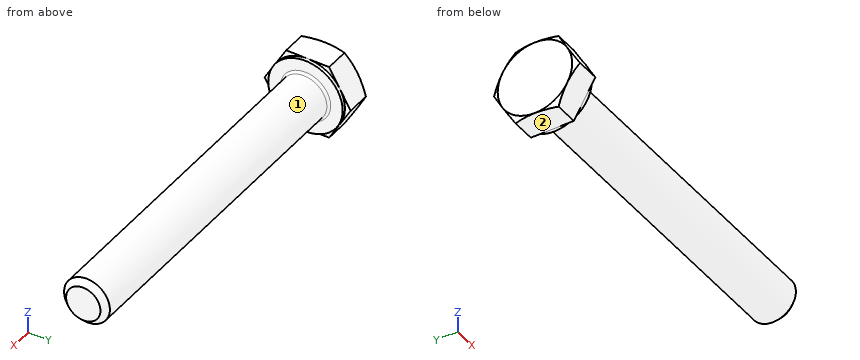
from build123d import *

# Parameters (mm, degrees)
BASE_EXTRUDE_DEPTH = 5.3
SKETCH4_W          = 0.6
SKETCH4_H          = 11.005553499
CHAMFER_2_SIZE     = 1
FILLET_2_R         = 0.4


with BuildPart() as part:
    # Sketch1 → Base-Extrude (new body)
    with BuildSketch(Plane(origin=(0, 0, 0), x_dir=(0, 0, -1), z_dir=(1, 0, 0))):
        Polygon((6.5, 3.75277675), (6.5, -3.75277675), (0, -7.505553499), (-6.5, -3.75277675), (-6.5, 3.75277675), (0, 7.505553499), align=None)
    extrude(amount=BASE_EXTRUDE_DEPTH)

    # Sketch2 → Boss-Revolve1 (revolve)
    with BuildSketch(Plane.XY, mode=Mode.PRIVATE) as boss_revolve1_sk:
        Polygon((0, 0), (65.3, 0), (65.3, 2.9175), (65.3, 4), (7.791693541, 4), (0, 4), align=None)
    revolve(boss_revolve1_sk.sketch.rotate(Axis((0, 0, 0), (1, 0, 0)), 90), axis=Axis((0, 0, 0), (1, 0, 0)))

    # Sketch3 → Cut-Revolve1 (revolve, cut)
    with BuildSketch(Plane.XY):
        Polygon((0, 6.5), (3.46730793, 12.505553499), (3.46730793, 17.505553499), (-10, 17.505553499), (-10, 6.5), align=None)
    revolve(axis=Axis((0, 0, 0), (1, 0, 0)), mode=Mode.SUBTRACT)

    # Sketch5 → Cut-Revolve2 (revolve, cut)
    with BuildSketch(Plane.XY):
        Polygon((5.3, 6.5), (1.83269207, 12.505553499), (1.83269207, 17.505553499), (11.83269207, 17.505553499), (11.83269207, 6.5), align=None)
    revolve(axis=Axis((0, 0, 0), (1, 0, 0)), mode=Mode.SUBTRACT)

    # Sketch4 → Cut-Revolve3 (revolve, cut)
    with BuildSketch(Plane.XY, mode=Mode.PRIVATE) as cut_revolve3_sk:
        with Locations((5, 12.00277675)):
            Rectangle(SKETCH4_W, SKETCH4_H)
    revolve(cut_revolve3_sk.sketch.rotate(Axis((0, 0, 0), (1, 0, 0)), 270), axis=Axis((0, 0, 0), (1, 0, 0)), mode=Mode.SUBTRACT)

    # Chamfer 2
    chamfer_2_edges = [part.edges().sort_by_distance(p)[0] for p in [
        (65.3, 0, -4),
    ]]
    chamfer(chamfer_2_edges, length=CHAMFER_2_SIZE)

    # Fillet 2
    fillet_2_edges = [part.edges().sort_by_distance(p)[0] for p in [
        (5.3, 0, -4),
    ]]
    fillet(fillet_2_edges, radius=FILLET_2_R)


solid = part.part
Design review of the part built by this model. Coordinates are the model's own, in mm. Face numbers are marked on the shaded views. A direction names the side the tool comes from. Give positions to 0.01 mm unless a question says otherwise; leave off trailing zeros. Loops run counter-clockwise (first coordinate to the right, second up) from the corner with the lowest first, then second, coordinate; pieces in that order, holes last. Notation, with made-up numbers: M 57,-23.75 L 108,-23.75 A22 cw 108,1.25 Z; hole C -27,1.25 d6. An arc over 180 degrees is marked long. Write item = value, one per line.
Q1. For the marked faces 1 and 2, list the 3-axis set-ups (+Z, -Z, +X, -X, +Y, -Y) from which the entire face can be reached by the end or side of a thin tool; tool diameter is ignored.
Output values:
face_1 = +X
face_2 = -Z, +X, -X, +Y, -Y
Q2. We need section A-A (x = 20.5). Give the boundary of the cut face in (y, z), plus the area to 3 significant figures.
Output values:
outline = C 0,0 d8
area = 50.3 mm^2
Q3. Insertion check: pin 1 (2 mm diameter, centred on x = 55, y = 4, fed in from +Z); pin 2 (5 mm diameter, centred on x = 8, z = 2, fed in from -Y); pin 3 (5 mm diameter, centred on x = 22, y = 2.5, fed in from +Z). Each pin has a flat end and moves straight along its axis. Give the tip position at first contact, or say it passes through.
Output values:
pin_1 = 2.65
pin_2 = -4
pin_3 = 4
Q4. To check wall thickness, follow line 1 (X direction, y = 1.5, z = -5); line 2 (Y direction, x = 48, z = -0.25); line 3 (Y direction, x = 48, z = 3.5). State the ranges of each line that lie inside material, in increasing order. Write a range as [from, to].
Output values:
line_1 = [0, 5.3]
line_2 = [-3.99, 3.99]
line_3 = [-1.94, 1.94]
